Design review of the part built by this model. Coordinates are the model's own, in mm. A direction names the side the tool comes from. Round coordinates to 2 decimals unless told otherwise and drop trailing zeros. Loops run counter-clockwise (first coordinate to the right, second up) from the corner with the lowest first, then second, coordinate; pieces in that order, holes last. Notation, with made-up numbers: (41.5, -3) -> (49.5, -3) arc R8 cw to (49.5, 5) -> close; hole circle Ø6 at (-19, 76.5). An arc over 180 degrees is marked (long way). Answer as CSV lines item,"result". Start each with the question number.
```python
from build123d import *

# Parameters (mm, degrees)
SKETCH1_W           = 75
SKETCH1_H           = 12
BOSS_EXTRUDE1_DEPTH = 12
SKETCH2_OUTSIDE_W   = 29.38
SKETCH2_OUTSIDE_H   = 29.38
SKETCH2_OUTSIDE_R   = 2.5
CUT_EXTRUDE1_DEPTH  = 2


with BuildPart() as part:
    # Sketch1 → Boss-Extrude1 (new body)
    with BuildSketch(Plane.XY):
        Rectangle(SKETCH1_W, SKETCH1_H)
    extrude(amount=BOSS_EXTRUDE1_DEPTH)

    # Sketch2 outside → Cut-Extrude1 (cut)
    with BuildSketch(Plane(origin=(37.5, 0, 0), x_dir=(0, 0, -1), z_dir=(1, 0, 0))):
        with Locations((-6, 0)):
            Rectangle(SKETCH2_OUTSIDE_W, SKETCH2_OUTSIDE_H)
        with Locations((-6, 0)):
            Circle(SKETCH2_OUTSIDE_R, mode=Mode.SUBTRACT)
    extrude(amount=-CUT_EXTRUDE1_DEPTH, mode=Mode.SUBTRACT)


solid = part.part
```
Q1. Add section C-C, the plane z = 1. Give the boundary of the cut face in (x, y).
Q2. To check wall thickness, follow probe 1 along X at (y, z) = (4.75, 3.5). State the ranges of the line that lie inside material, in increasing order. Write a range as from..to.
Q3. Add section B-B, the plane z = 6. Give the boundary of the cut face in (x, y).
Q4. Add section A-A, the plane y = 0. Give the boundary of the cut face in (x, z), and give its area (3 significant figures).
Q5. Machinability: for faces 1 (the flat face through (35.5, 0, 9)), 2 (the flat face through (-2, 0, 0)), which of the approach directions +Z, -Z, +X, -X, +Y, -Y give a long, thin tool a straight path to every point of the face, cutting with its end or side? Answer none if there is none.
Q6. Add section D-D, the plane y = 5.25. Give the boundary of the cut face in (x, z).
Worked answers:
1,outline,"(-37.5, -6) -> (35.5, -6) -> (35.5, 6) -> (-37.5, 6) -> close"
2,probe 1,"x = -37.5..35.5"
3,outline,"(-37.5, -6) -> (35.5, -6) -> (35.5, -2.5) -> (37.5, -2.5) -> (37.5, 2.5) -> (35.5, 2.5) -> (35.5, 6) -> (-37.5, 6) -> close"
4,outline,"(-37.5, 0) -> (35.5, 0) -> (35.5, 3.5) -> (37.5, 3.5) -> (37.5, 8.5) -> (35.5, 8.5) -> (35.5, 12) -> (-37.5, 12) -> close"
4,area,"886 mm^2"
5,face 1,"+X"
5,face 2,"-Z, +X, -X, +Y, -Y"
6,outline,"(-37.5, 0) -> (35.5, 0) -> (35.5, 12) -> (-37.5, 12) -> close"
